Geometry: final body of the model. Coordinates: model frame, mm. A direction names the side the tool comes from. Round coordinates to 2 decimals unless told otherwise and drop trailing zeros. Loops run counter-clockwise (first coordinate to the right, second up) from the corner with the lowest first, then second, coordinate; pieces in that order, holes last. Notation, with made-up numbers: (27, 10) - (60, 10) arc R13 cw to (60, 28) - close; hole circle Ø1 at (53.25, 10.25). An arc over 180 degrees is marked (long way). Answer in a Markdown table with one row per item. Add a question column.
from build123d import *

# Parameters (mm, degrees)
FLANGE_PLATE_125X125X16_DEPTH = 16
BOLT_HOLES_SKETCH_R           = 7.5
BOLT_HOLES_4X_15_DEPTH        = 16
HUB_SKETCH_R                  = 34
HUB_68X54_DEPTH               = 54
HUB_CHAMFER_2X45_SIZE         = 2
BORE_SKETCH_R                 = 14
BORE_28_DEPTH                 = 54
BORE_CHAMFER_2X45_SIZE        = 2


with BuildPart() as part:
    # Flange Plate Sketch → Flange Plate 125x125x16 (new body)
    with BuildSketch(Plane.XY):
        with BuildLine():
            Line((16, 0), (109, 0))
            ThreePointArc((109, 0), (120.313708499, -4.686291501), (125, -16))
            Line((125, -16), (125, -109))
            ThreePointArc((125, -109), (120.313708499, -120.313708499), (109, -125))
            Line((109, -125), (16, -125))
            ThreePointArc((16, -125), (4.686291501, -120.313708499), (0, -109))
            Line((0, -109), (0, -16))
            ThreePointArc((0, -16), (4.686291501, -4.686291501), (16, 0))
        make_face()
    extrude(amount=FLANGE_PLATE_125X125X16_DEPTH)

    # Bolt Holes Sketch → Bolt Holes 4xØ15 (cut)
    with BuildSketch(Plane.XY.offset(16)):
        with Locations((16, -16)):
            Circle(BOLT_HOLES_SKETCH_R)
        with Locations((109, -16)):
            Circle(BOLT_HOLES_SKETCH_R)
        with Locations((109, -109)):
            Circle(BOLT_HOLES_SKETCH_R)
        with Locations((16, -109)):
            Circle(BOLT_HOLES_SKETCH_R)
    extrude(amount=-BOLT_HOLES_4X_15_DEPTH, mode=Mode.SUBTRACT)

    # Hub Sketch → Hub Ø68x54 (add)
    with BuildSketch(Plane.XY.offset(16)):
        with Locations((62.5, -62.5)):
            Circle(HUB_SKETCH_R)
    extrude(amount=HUB_68X54_DEPTH)

    # Hub Chamfer 2x45
    hub_chamfer_2x45_edges = [part.edges().sort_by_distance(p)[0] for p in [
        (28.5, -62.5, 16),
    ]]
    chamfer(hub_chamfer_2x45_edges, length=HUB_CHAMFER_2X45_SIZE)

    # Bore Sketch → Bore Ø28 (cut)
    with BuildSketch(Plane.XY.offset(70)):
        with Locations((62.5, -62.5)):
            Circle(BORE_SKETCH_R)
    extrude(amount=-BORE_28_DEPTH, mode=Mode.SUBTRACT)

    # Bore Chamfer 2x45
    bore_chamfer_2x45_edges = [part.edges().sort_by_distance(p)[0] for p in [
        (48.5, -62.5, 70),
    ]]
    chamfer(bore_chamfer_2x45_edges, length=BORE_CHAMFER_2X45_SIZE)


solid = part.part
1) Pull-direction query (X, two-part tool) for faces 3 (the cylindrical face through (14.37, -116.32, 8.11)), 4 (the flat face through (77, -70, 70)), 5 (the cylindrical face through (4.811, -120.437, 7.888)); classes: pulls with the +X half, pulls with the -X half, needs draft (parallel to the pull), parting line crosses it, or undercut.
2) Section C-C, the plane z = 24. Return the cut outline in (x, y).
3) Section A-A, the plane x = 111. Return the cut outline in (y, z).
4) Contact query for flat-ended pins moving along their axis: pin 1 Ø24 at (x, y) = (109, -109) entering from +Z; pin 2 Ø12 at (x, y) = (16, -16) entering from +Z; pin 3 Ø12 at (x, z) = (33.5, 32.5) entering from -Y; pin 4 Ø1 at (y, z) = (-39.5, 31.5) entering from -X. Output: stop coordinate, or through.
5) Reachability of faces 1 (the cylindrical face through (120.189, -4.563, 7.888)), 2 (the flat face through (36, -89, 16)) from +Z, -Z, +X, -X, +Y, -Y: full face, straight path, thin tool, end or side. Return the list, or none.
6) Section D-D, the plane x = 62.5. Return the cut outline in (y, z).
7) Section B-B, the plane y = -62.5. Return the cut outline in (x, z).
8) Material intervals for line 1 along Y through (x, z) = (109, 3.25); line 2 along Y through (x, z) = (62.5, 47); line 3 along Z through (x, y) = (34, -24), sorted ascending. Write a range as from..to.
Evaluation:
| question | item | result |
|---|---|---|
| 1 | face 3 | undercut |
| 1 | face 4 | needs draft |
| 1 | face 5 | pulls with the -X half |
| 2 | outline | circle Ø68 at (62.5, -62.5); hole circle Ø28 at (62.5, -62.5) |
| 3 | outline | (-124.87, 0) - (-116.23, 0) - (-116.23, 16) - (-124.87, 16) - close; (-101.77, 0) - (-23.23, 0) - (-23.23, 16) - (-101.77, 16) - close; (-8.77, 0) - (-0.13, 0) - (-0.13, 16) - (-8.77, 16) - close |
| 4 | pin 1 | stops at z = 16 |
| 4 | pin 2 | passes through |
| 4 | pin 3 | stops at y = -87.54 |
| 4 | pin 4 | stops at x = 37.01 |
| 5 | face 1 | +Z, -Z, +X, +Y |
| 5 | face 2 | +Z |
| 6 | outline | (-125, 0) - (0, 0) - (0, 16) - (-26.5, 16) - (-28.5, 18) - (-28.5, 70) - (-46.5, 70) - (-48.5, 68) - (-48.5, 16) - (-76.5, 16) - (-76.5, 68) - (-78.5, 70) - (-96.5, 70) - (-96.5, 18) - (-98.5, 16) - (-125, 16) - close |
| 7 | outline | (0, 0) - (125, 0) - (125, 16) - (98.5, 16) - (96.5, 18) - (96.5, 70) - (78.5, 70) - (76.5, 68) - (76.5, 16) - (48.5, 16) - (48.5, 68) - (46.5, 70) - (28.5, 70) - (28.5, 18) - (26.5, 16) - (0, 16) - close |
| 8 | line 1 | y = -125..-116.5, -101.5..-23.5, -8.5..0 |
| 8 | line 2 | y = -96.5..-76.5, -48.5..-28.5 |
| 8 | line 3 | z = 0..16 |
